Could you check a few things on this drawing? It's one solid part, dimensions in mm from its lowest x, y, z. A direction names the side the tool comes from. Round coordinates to 2 decimals unless told otherwise and drop trailing zeros. Loops run counter-clockwise (first coordinate to the right, second up) from the corner with the lowest first, then second, coordinate; pieces in that order, holes last. Notation, with made-up numbers: (-25, 71.25) -> (31, 71.25) arc R6 ccw to (31, 76.25) -> close; hole circle Ø4 at (68.25, 83.5). An arc over 180 degrees is marked (long way). Use one line per item in the form item = value. Start each with the question number.
Item 1: If we section it at C-C (x = 34.5): Write out the boundary of the cut face in (y, z).
Item 2: If I drill on L1, parallel to Y at x = 9.5, z = 7; L2, parallel to Z at x = 30.5, y = 9; L3, parallel to Y at x = 19, z = 10.75, over which ranges is the centre line in solid material (lowest first)? Write a range as [from, to].
Item 3: I'm going to push flat-ended pins straight in: pin 1 Ø6 at (x, y) = (35, 5.5) entering from +Z; pin 2 Ø1 at (x, y) = (26.5, 9.5) entering from +Z; pin 3 Ø1 at (x, z) = (7, 7) entering from +Y. Where does each tip first touch, or does it pass through?
Item 4: If we section it at A-A (y = 7): Write out the boundary of the cut face in (x, z), then the cut area to 3 significant figures.
Item 5: For the marked faces 1 and 2, which set-ups out of +Z, -Z, +X, -X, +Y, -Y let a thin tool reach every point of the face, with its end or its side?
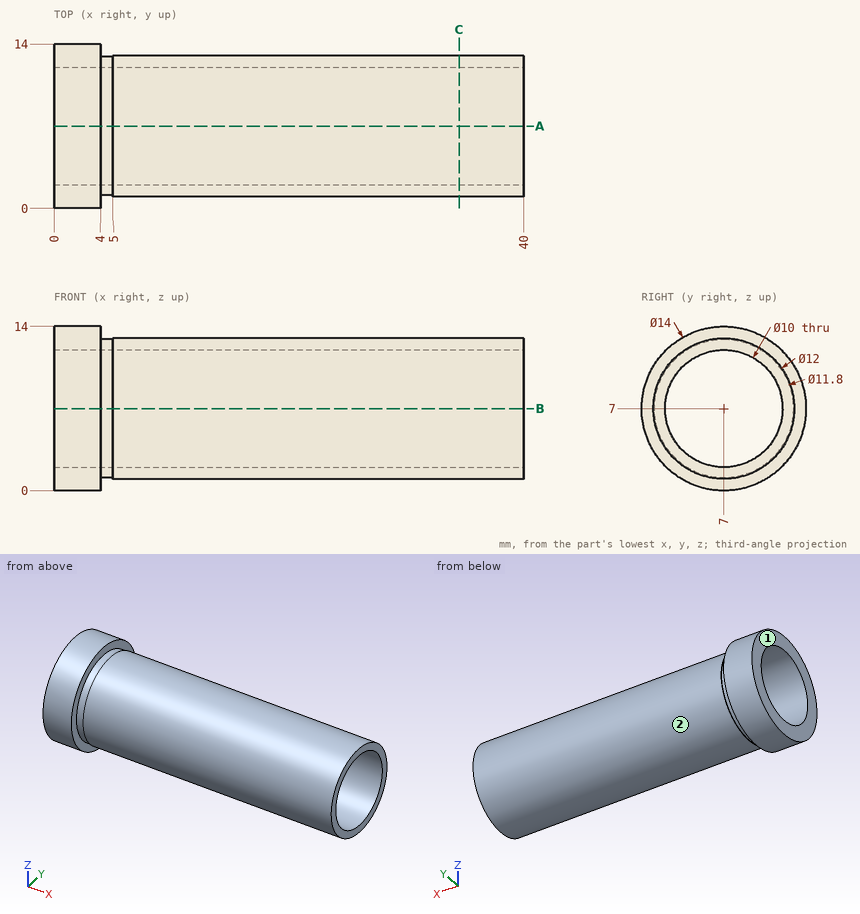
Values found:
q1.outline = circle Ø12 at (7, 7); hole circle Ø10 at (7, 7)
q2.L1 = [1, 2], [12, 13]
q2.L2 = [1.34, 2.42], [11.58, 12.66]
q2.L3 = [2.32, 3.69], [10.31, 11.68]
q3.pin_1 = 13
q3.pin_2 = 12.66
q3.pin_3 = 13
q4.outline = (0, 0) -> (4, 0) -> (4, 1.1) -> (5, 1.1) -> (5, 1) -> (40, 1) -> (40, 2) -> (0, 2) -> close; (0, 12) -> (40, 12) -> (40, 13) -> (5, 13) -> (5, 12.9) -> (4, 12.9) -> (4, 14) -> (0, 14) -> close
q4.area = 87.8 mm2
q5.face_1 = +Z, -Z, -X, +Y, -Y
q5.face_2 = +X
